from build123d import *

# Parameters (mm, degrees)
BOSS_EXTRUDE1_DEPTH = 500


with BuildPart() as part:
    # Sketch1 → Boss-Extrude1 (new body)
    with BuildSketch(Plane.XY):
        with BuildLine():
            Line((-10, -13.2), (-6.5, -13.2))
            Line((-6.5, -13.2), (-6.5, -15))
            Line((-6.5, -15), (-10, -15))
            ThreePointArc((-10, -15), (-14.242640687, -13.242640687), (-16, -9))
            Line((-16, -9), (-16, 9))
            ThreePointArc((-16, 9), (-14.242640687, 13.242640687), (-10, 15))
            Line((-10, 15), (10, 15))
            ThreePointArc((10, 15), (14.242640687, 13.242640687), (16, 9))
            Line((16, 9), (16, -9))
            ThreePointArc((16, -9), (14.242640687, -13.242640687), (10, -15))
            Line((10, -15), (6.5, -15))
            Line((6.5, -15), (6.5, -13.2))
            Line((6.5, -13.2), (10, -13.2))
            ThreePointArc((10, -13.2), (12.969848481, -11.969848481), (14.2, -9))
            Line((14.2, -9), (14.2, 9))
            ThreePointArc((14.2, 9), (12.969848481, 11.969848481), (10, 13.2))
            Line((10, 13.2), (-10, 13.2))
            ThreePointArc((-10, 13.2), (-12.969848481, 11.969848481), (-14.2, 9))
            Line((-14.2, 9), (-14.2, -9))
            ThreePointArc((-14.2, -9), (-12.969848481, -11.969848481), (-10, -13.2))
        make_face()
    extrude(amount=BOSS_EXTRUDE1_DEPTH)


solid = part.part
Can you work these out from the model? Positions are in its coordinate system, mm. A direction names the side the tool comes from. Give positions to 0.01 mm unless a question says otherwise; leave off trailing zeros. Loops run counter-clockwise (first coordinate to the right, second up) from the corner with the lowest first, then second, coordinate; pieces in that order, holes last. Notation, with made-up numbers: (66.25, 1) - (106.25, 1) arc R30 ccw to (106.25, 29) - close; hole circle Ø10 at (-30.5, 85). An arc over 180 degrees is marked (long way). Answer as a JSON object with one key per item and string values.
Q1. Imagine slicing it at C-C on x = 1. Write out the boundary of the cut face in (y, z).
Geometry says:
{"outline": "(13.2, 0) - (15, 0) - (15, 500) - (13.2, 500) - close"}
Q2. Imagine slicing it at B-B on z = 389.5. Write out the boundary of the cut face in (x, y).
Geometry says:
{"outline": "(-16, -9) arc R6 ccw to (-10, -15) - (-6.5, -15) - (-6.5, -13.2) - (-10, -13.2) arc R4.2 cw to (-14.2, -9) - (-14.2, 9) arc R4.2 cw to (-10, 13.2) - (10, 13.2) arc R4.2 cw to (14.2, 9) - (14.2, -9) arc R4.2 cw to (10, -13.2) - (6.5, -13.2) - (6.5, -15) - (10, -15) arc R6 ccw to (16, -9) - (16, 9) arc R6 ccw to (10, 15) - (-10, 15) arc R6 ccw to (-16, 9) - close"}
Q3. Imagine slicing it at A-A on y = 3.5. Write out the boundary of the cut face in (x, z), plus the area to 3 significant figures.
Geometry says:
{"outline": "(-16, 0) - (-14.2, 0) - (-14.2, 500) - (-16, 500) - close; (14.2, 0) - (16, 0) - (16, 500) - (14.2, 500) - close", "area": "1,800 mm²"}
Q4. If we mould it in two halves opening along Y, with no side actions, what happens to faces 3 (the flat face through (1.3, 13.4, 500)), 4 (the flat face through (0, 15, 246)), 5 (the flat face through (14.2, 0, 246)), 6 (the flat face through (-14.2, 0, 246))? For each: pulls with the +Y half, pulls with the -Y half, needs draft (parallel to the pull), parting line crosses it, or undercut.
Geometry says:
{"face 3": "needs draft", "face 4": "pulls with the +Y half", "face 5": "undercut", "face 6": "undercut"}
Q5. Will these pins go through, and if not, where does the flat tip stop? P1, Ø0.9, axis at y = -14, z = 191.5, coming from the -X side; P2, Ø1.5, axis at x = 12.5, z = 312.5, coming from the -Y side; P3, Ø2, axis at y = -14.5, z = 253.5, coming from the +X side.
Geometry says:
{"P1": "x = -13.91", "P2": "y = -14.74", "P3": "x = 13.97"}
Q6. If I drill on L1, parallel to X at y = -13.25, z = 147.5; L2, parallel to X at y = -3.5, z = 236; L3, parallel to Y at x = 6, z = 101, over which ranges is the centre line in solid material (lowest first)?
Geometry says:
{"L1": "-14.24 to -6.5, 6.5 to 14.24", "L2": "-16 to -14.2, 14.2 to 16", "L3": "13.2 to 15"}
Q7. Which directions (+Z, -Z, +X, -X, +Y, -Y) give clear straight access to the entire face, cutting with the end or side of a thin tool? Please do faces 1 (the flat face through (1.3, 13.4, 0)), 2 (the flat face through (0, 13.2, 246)).
Geometry says:
{"face 1": "-Z, +X, -X, +Y, -Y", "face 2": "+Z, -Z"}
